```python
from build123d import *

# Parameters (mm, degrees)
BOSS_EXTRUDE1_DEPTH                                 = 75
HOLE_SIZE_BY_SOCKET_HEAD_CAP_SCREW_TYPE_D           = 4.5
HOLE_SIZE_BY_SOCKET_HEAD_CAP_SCREW_TYPE_CBORE_D     = 8
HOLE_SIZE_BY_SOCKET_HEAD_CAP_SCREW_TYPE_CBORE_DEPTH = 4.6
M5_TAPPED_HOLE1_D                                   = 4.2
M5_TAPPED_HOLE1_DEPTH                               = 12.4
M5_TAPPED_HOLE1_TIP                                 = 1.2618073
M5_TAPPED_HOLE2_D                                   = 4.2
M5_TAPPED_HOLE2_DEPTH                               = 12.4
M5_TAPPED_HOLE2_TIP                                 = 1.2618073
CHAMFER1_SIZE                                       = 1
SIZE_MM_BLIND_PIN_HOLE1_D                           = 5
SIZE_MM_BLIND_PIN_HOLE1_DEPTH                       = 7.5
SIZE_MM_BLIND_PIN_HOLE1_TIP                         = 1.502151548


with BuildPart() as part:
    # Sketch1 → Boss-Extrude1 (new, symmetric)
    with BuildSketch(Plane.XY):
        Polygon((0, 0), (0, 32), (-38, 32), (-38, 2), (-2, 2), (-2, 0), align=None)
    extrude(amount=BOSS_EXTRUDE1_DEPTH, both=True)

    # Hole Size (by socket head cap screw type)1 (through all)
    with Locations(Plane(origin=(0, 32, 0), x_dir=(1, 0, 0), z_dir=(0, 1, 0))):
        with Locations((-32, -68.3), (-32, 68.3), (-6, 42.3), (-32, 42.3), (-6, 68.3), (-6, -68.3), (-6, -42.3), (-32, -42.3)):
            CounterBoreHole(HOLE_SIZE_BY_SOCKET_HEAD_CAP_SCREW_TYPE_D / 2, HOLE_SIZE_BY_SOCKET_HEAD_CAP_SCREW_TYPE_CBORE_D / 2, HOLE_SIZE_BY_SOCKET_HEAD_CAP_SCREW_TYPE_CBORE_DEPTH)

    # M5 Tapped Hole1
    with Locations(Plane(origin=(-38, 0, 0), x_dir=(0, 0, -1), z_dir=(-1, 0, 0))):
        with Locations((0, -17), (-20, -17), (20, -17)):
            Hole(M5_TAPPED_HOLE1_D / 2, depth=M5_TAPPED_HOLE1_DEPTH)
            with Locations((0, 0, -(M5_TAPPED_HOLE1_DEPTH + M5_TAPPED_HOLE1_TIP / 2))):  # 118° drill point
                Cone(0, M5_TAPPED_HOLE1_D / 2, M5_TAPPED_HOLE1_TIP, mode=Mode.SUBTRACT)

    # M5 Tapped Hole2
    with Locations(Plane(origin=(0, 32, 0), x_dir=(1, 0, 0), z_dir=(0, 1, 0))):
        with Locations((-19, -16.3), (-19, 68.3), (-19, 42.3), (-19, -42.3), (-19, -68.3), (-19, 16.3)):
            Hole(M5_TAPPED_HOLE2_D / 2, depth=M5_TAPPED_HOLE2_DEPTH)
            with Locations((0, 0, -(M5_TAPPED_HOLE2_DEPTH + M5_TAPPED_HOLE2_TIP / 2))):  # 118° drill point
                Cone(0, M5_TAPPED_HOLE2_D / 2, M5_TAPPED_HOLE2_TIP, mode=Mode.SUBTRACT)

    # Chamfer1
    chamfer1_edges = [part.edges().sort_by_distance(p)[0] for p in [
        (-38, 17, 75),
        (-38, 17, -75),
        (0, 16, -75),
        (0, 16, 75),
    ]]
    chamfer(chamfer1_edges, length=CHAMFER1_SIZE)

    # Size mm Blind Pin Hole1
    with Locations(Plane(origin=(0, 32, 0), x_dir=(1, 0, 0), z_dir=(0, 1, 0))):
        with Locations((-19, 0)):
            Hole(SIZE_MM_BLIND_PIN_HOLE1_D / 2, depth=SIZE_MM_BLIND_PIN_HOLE1_DEPTH)
            with Locations((0, 0, -(SIZE_MM_BLIND_PIN_HOLE1_DEPTH + SIZE_MM_BLIND_PIN_HOLE1_TIP / 2))):  # 118° drill point
                Cone(0, SIZE_MM_BLIND_PIN_HOLE1_D / 2, SIZE_MM_BLIND_PIN_HOLE1_TIP, mode=Mode.SUBTRACT)


solid = part.part
```
Geometry check sheet. Reference: the model listing, model coordinates, mm. A direction names the side the tool comes from. Give positions to 0.01 mm unless a question says otherwise; leave off trailing zeros. One line per question, with ' | ' between items.
Item 1: Access from +Z, -Z, +X, -X, +Y, -Y to the whole of each face (thin tool, end or side, straight path). Record for faces 4 (the cylindrical face through (-31.71, 15.23, -18.87)), 5 (the cylindrical face through (-21.003, 25.713, -16.931)), 6 (the flat face through (-15, 32, 1)).
Determined:
face 4: -X | face 5: +Y | face 6: +Z, -Z, +X, -X, +Y
Item 2: Sectioned sample at A-A, the plane y = 8. State how many separate pieces and enclosed holes the cut face has, plus the area to 3 significant figures.
Determined:
separate pieces: 1 | enclosed holes: 8 | area: 5,570 mm^2
Item 3: Draft check along Y on faces 1 (the flat face through (0, 16, 1)), 2 (the flat face through (-4, 27.4, 44)), 3 (the conical face through (-24.56, 16.75, -19.73)). Enter one of: released by +Y, released by -Y, zero draft, split by the parting line, or undercut.
Determined:
face 1: zero draft | face 2: released by +Y | face 3: undercut
Item 4: Scan lines: line 1 along X through (y, z) = (29, 42.3); line 2 along Z through (x, y) = (-29, 17); line 3 along X through (y, z) = (5, 43). Record each from-to range of solid material in increasing order.
Determined:
line 1: -38 to -36, -28 to -21.1, -16.9 to -10, -2 to 0 | line 2: -75 to -22.1, -17.9 to -2.1, 2.1 to 17.9, 22.1 to 75 | line 3: -38 to -34.14, -29.86 to -8.14, -3.86 to 0
Item 5: Depth check by flat-ended pin: pin 1 (3.5 mm diameter, centred on x = -19, z = -42.3, fed in from -Y); pin 2 (5 mm diameter, centred on x = -32, z = -42.3, fed in from +Y); pin 3 (3.5 mm diameter, centred on x = -19, z = -16.3, fed in from +Y); pin 4 (2.5 mm diameter, centred on x = -6.5, z = 42.5, fed in from +Y). Enter the tip coordinate at first touch or a pass-through.
Determined:
pin 1: y = 2 | pin 2: y = 27.4 | pin 3: y = 19.39 | pin 4: through
